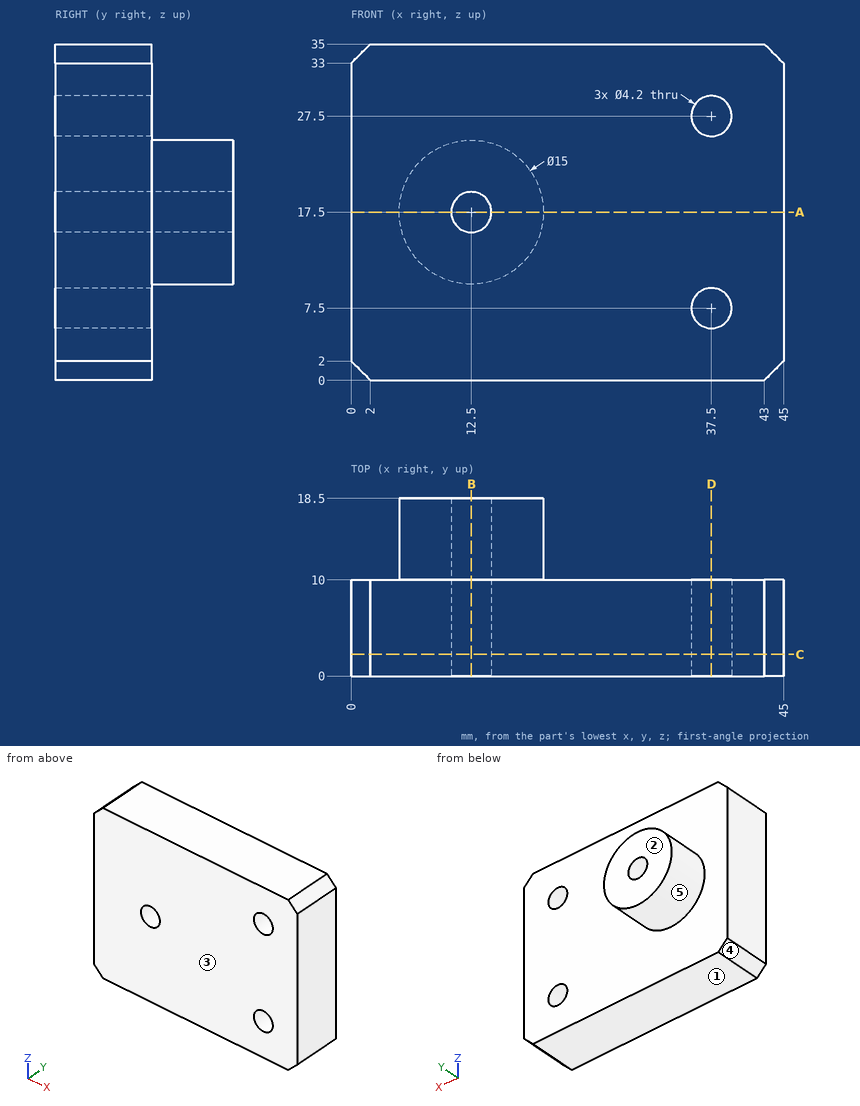
Drawing for the job (mm, zero at the part's lowest x, y, z). A direction names the side the tool comes from. Give positions to 0.01 mm unless a question says otherwise; leave off trailing zeros. Order: outer loops, then holes, each group sorted by start corner. A loop starts at its lowest first (then second) coordinate and runs counter-clockwise, first axis right, second up. Notation, with made-up numbers: M 54,6.5 L 59,6.5 A29 cw 59,38.5 Z; hole C 33.25,52.25 d11. An arc over 180 degrees is marked long. Put each result on its own line as item: value. Start each with the question number.
(1) Drill centre lines: line 1 along Z through (x, y) = (37.5, 5); line 2 along Z through (x, y) = (12.5, 8.5); line 3 along X through (y, z) = (17.75, 17.5). Where is each one in solid material? Low to high.
(2) Saw through at A-A, the plane z = 17.5. Write the cut outline in (x, y).
(3) Saw through at D-D, the plane x = 37.5. Write the cut outline in (y, z).
(4) Saw through at C-C, the plane y = 2.25. Write the cut outline in (x, z), then the cut area to 3 significant figures.
(5) Mould opens along Y. For the marked faces 1, 2 and 3 say: +Y half, -Y half, draft (parallel to the pull), parting line (faces both ways), or undercut.
(6) Saw through at B-B, the plane x = 12.5. Write the cut outline in (y, z), then the cut area to 3 significant figures.
(7) Which spindle directions (+Z, -Z, +X, -X, +Y, -Y) get a long thin tool onto all of the face, cutting with end or side? Do the marked faces 4 and 5. Say none if no direction does.
(8) Flat gauge pins, fed straight in: pin 1 Ø6.5 at (x, z) = (37.5, 27.5) entering from -Y; pin 2 Ø2 at (x, z) = (26, 24.5) entering from +Y; pin 3 Ø3.5 at (x, z) = (37.5, 7.5) entering from +Y. Where does each tip first touch, or does it go through?
Check result:
1. line 1: z = 0 to 5.4, 9.6 to 25.4, 29.6 to 35
1. line 2: z = 0 to 15.4, 19.6 to 35
1. line 3: x = 5 to 10.4, 14.6 to 20
2. outline: M 0,0 L 10.4,0 L 10.4,18.5 L 5,18.5 L 5,10 L 0,10 Z; M 14.6,0 L 45,0 L 45,10 L 20,10 L 20,18.5 L 14.6,18.5 Z
3. outline: M 0,0 L 10,0 L 10,5.4 L 0,5.4 Z; M 0,9.6 L 10,9.6 L 10,25.4 L 0,25.4 Z; M 0,29.6 L 10,29.6 L 10,35 L 0,35 Z
4. outline: M 0,2 L 2,0 L 43,0 L 45,2 L 45,33 L 43,35 L 2,35 L 0,33 Z; hole C 12.5,17.5 d4.2; hole C 37.5,7.5 d4.2; hole C 37.5,27.5 d4.2
4. area: 1,530 mm2
5. face 1: draft
5. face 2: +Y half
5. face 3: -Y half
6. outline: M 0,0 L 10,0 L 10,10 L 18.5,10 L 18.5,15.4 L 0,15.4 Z; M 0,19.6 L 18.5,19.6 L 18.5,25 L 10,25 L 10,35 L 0,35 Z
6. area: 400 mm2
7. face 4: -Z, -X, +Y, -Y
7. face 5: +Y
8. pin 1: stops at y = 0
8. pin 2: stops at y = 10
8. pin 3: passes through
